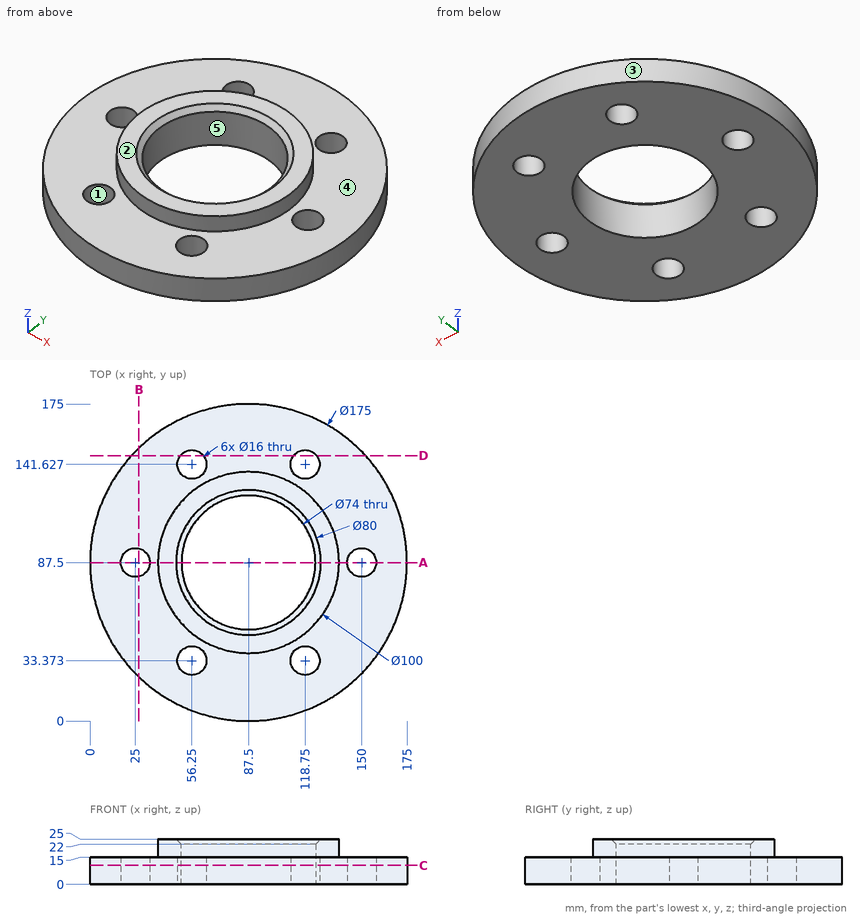
Could you check a few things on this drawing? It's one solid part, dimensions in mm from its lowest x, y, z. A direction names the side the tool comes from. Give positions to 0.01 mm unless a question says otherwise; leave off trailing zeros. Order: outer loops, then holes, each group sorted by start corner. A loop starts at its lowest first (then second) coordinate and runs counter-clockwise, first axis right, second up. Notation, with made-up numbers: (-30.75, 52.25) -> (-11.75, 52.25) arc R19 ccw to (-11.75, 73.25) -> close; hole circle Ø4 at (12, 74.5). An arc over 180 degrees is marked (long way). Answer in a Markdown table with one row per item. Add a question column.
Item 1: Imagine slicing it at C-C (z = 10.5). List the corners of the cut face in (x, y) for me.
Item 2: Imagine slicing it at B-B (x = 27). List the corners of the cut face in (y, z) for me, and give its area (3 significant figures).
Item 3: I'm going to push flat-ended pins straight in: P1, Ø3, axis at x = 118, z = 18, coming from the +Y side; P2, Ø12, axis at x = 47, z = 19.5, coming from the +Y side; P3, Ø4, axis at x = 142.5, z = 14.5, coming from the -Y side. Where does each tip first touch, or does it pass through?
Item 4: Please list where these lines run through material, in increasing order: probe 1 along Y at (x, z) = (56.25, 4.25) (1 decimal); probe 2 along Y at (x, z) = (87.5, 13); probe 3 along X at (y, z) = (91.5, 5).
Item 5: We'd pull the mould along X, two halves only. Please class the marked faces 1, 2 and 3: pulls with the +X half, pulls with the -X half, needs draft (parallel to the pull), parting line crosses it, or undercut.
Item 6: For the marked faces 4 and 5, which set-ups out of +Z, -Z, +X, -X, +Y, -Y let a thin tool reach every point of the face, with its end or its side?
Item 7: Imagine slicing it at D-D (y = 146.5). List the corners of the cut face in (x, z) for me (1 decimal), and give its area (3 significant figures).
Item 8: Imagine slicing it at A-A (y = 87.5). List the corners of the cut face in (x, z) for me, and give its area (3 significant figures).
Result:
| question | item | result |
|---|---|---|
| 1 | outline | circle Ø175 at (87.5, 87.5); hole circle Ø16 at (25, 87.5); hole circle Ø16 at (56.25, 33.37); hole circle Ø16 at (56.25, 141.63); hole circle Ø74 at (87.5, 87.5); hole circle Ø16 at (118.75, 33.37); hole circle Ø16 at (118.75, 141.63); hole circle Ø16 at (150, 87.5) |
| 2 | outline | (24.29, 0) -> (79.75, 0) -> (79.75, 15) -> (24.29, 15) -> close; (95.25, 0) -> (150.71, 0) -> (150.71, 15) -> (95.25, 15) -> close |
| 2 | area | 1,660 mm2 |
| 3 | P1 | y = 128.23 |
| 3 | P2 | y = 167.01 |
| 3 | P3 | y = 17.88 |
| 4 | probe 1 | 5.8 to 25.4, 41.4 to 67.7, 107.3 to 133.6, 149.6 to 169.2 |
| 4 | probe 2 | 0 to 50.5, 124.5 to 175 |
| 4 | probe 3 | 0.09 to 18.07, 31.93 to 50.72, 124.28 to 143.07, 156.93 to 174.91 |
| 5 | face 1 | undercut |
| 5 | face 2 | needs draft |
| 5 | face 3 | parting line crosses it |
| 6 | face 4 | +Z |
| 6 | face 5 | +Z, -Z |
| 7 | outline | (22.9, 0) -> (49.9, 0) -> (49.9, 15) -> (22.9, 15) -> close; (62.6, 0) -> (112.4, 0) -> (112.4, 15) -> (62.6, 15) -> close; (125.1, 0) -> (152.1, 0) -> (152.1, 15) -> (125.1, 15) -> close |
| 7 | area | 1,560 mm2 |
| 8 | outline | (0, 0) -> (17, 0) -> (17, 15) -> (0, 15) -> close; (33, 0) -> (50.5, 0) -> (50.5, 22) -> (47.5, 25) -> (37.5, 25) -> (37.5, 15) -> (33, 15) -> close; (124.5, 0) -> (142, 0) -> (142, 15) -> (137.5, 15) -> (137.5, 25) -> (127.5, 25) -> (124.5, 22) -> close; (158, 0) -> (175, 0) -> (175, 15) -> (158, 15) -> close |
| 8 | area | 1,290 mm2 |
